Design review of the part shown in the three views and the two pictorial views. Dimensions are in mm from the part's minimum x, y and z. A direction names the side the tool comes from. Round coordinates to 2 decimals unless told otherwise and drop trailing zeros. Order: outer loops, then holes, each group sorted by start corner. A loop starts at its lowest first (then second) coordinate and runs counter-clockwise, first axis right, second up.
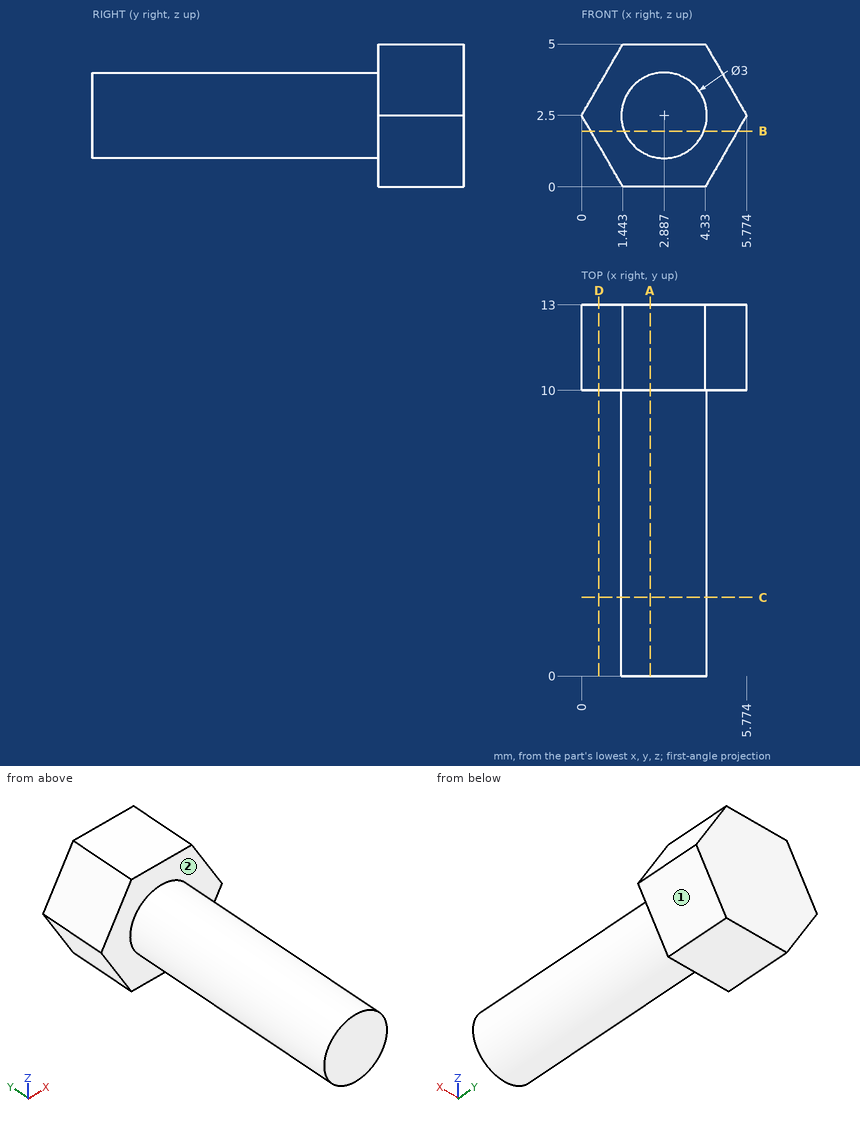
1) Take a section at C-C on y = 2.75. Give the boundary of the cut face in (x, z).
Results:
outline: circle Ø3 at (2.89, 2.5)
2) To check wall thickness, follow line 1 along Y through (x, z) = (3.5, 4.5); line 2 along Z through (x, y) = (2.9, 5); line 3 along Z through (x, y) = (4.5, 12.5) (1 decimal). State the ranges of each line that lie inside material, in increasing order.
Results:
line 1: y = 10 to 13
line 2: z = 1 to 4
line 3: z = 0.3 to 4.7
3) Take a section at D-D on x = 0.6. Give the boundary of the cut face in (y, z).
Results:
outline: (10, 1.46) - (13, 1.46) - (13, 3.54) - (10, 3.54) - close
4) Take a section at B-B on z = 1.95. Give the boundary of the cut face in (x, y) (1 decimal).
Results:
outline: (0.3, 10) - (1.5, 10) - (1.5, 0) - (4.3, 0) - (4.3, 10) - (5.5, 10) - (5.5, 13) - (0.3, 13) - close
5) For the marked faces 1 and 2, list the 3-axis set-ups (+Z, -Z, +X, -X, +Y, -Y) from which the entire face can be reached by the end or side of a thin tool; tool diameter is ignored.
Results:
face 1: -Z, +X, +Y, -Y
face 2: -Y
6) Take a section at A-A on x = 2.4. Give the boundary of the cut face in (y, z).
Results:
outline: (0, 1.08) - (10, 1.08) - (10, 0) - (13, 0) - (13, 5) - (10, 5) - (10, 3.92) - (0, 3.92) - close
7) Clearance check with flat-ended pins moving along their axes: P1, Ø1.5, axis at x = 0.5, z = 2, coming from the -Y side; P2, Ø2, axis at x = 4, y = 6, coming from the +Z side. State where each tip first meets the part, or that it passes through.
Results:
P1: stops at y = 10
P2: stops at z = 4
